Source: three-view drawing plus pictorial views. Frame: mm from the lowest corner of the part. Give positions to 0.01 mm unless a question says otherwise; leave off trailing zeros. Loops run counter-clockwise (first coordinate to the right, second up) from the corner with the lowest first, then second, coordinate; pieces in that order, holes last. Notation, with made-up numbers: M -40,67.5 L -24,67.5 A28 ccw -24,86.5 Z; hole C 53,56 d7. An arc over 180 degrees is marked long. Answer as a JSON object with one key per item and string values. Group by question number.
1) Section query C-C on y = 10. Return loops of the section in (x, z).
2) Section query A-A on z = 352. Return loops of the section in (x, y), plus the area to 3 significant figures.
3) Ray query, L1, parallel to X at y = 13.5, z = 229.5; L2, parallel to Z at x = 1394, y = 34; L3, parallel to Z at x = 262, y = 25.5. Return the intervals inside material, ascending.
4) Section query B-B on x = 1876.5. Return loops of the section in (y, z).
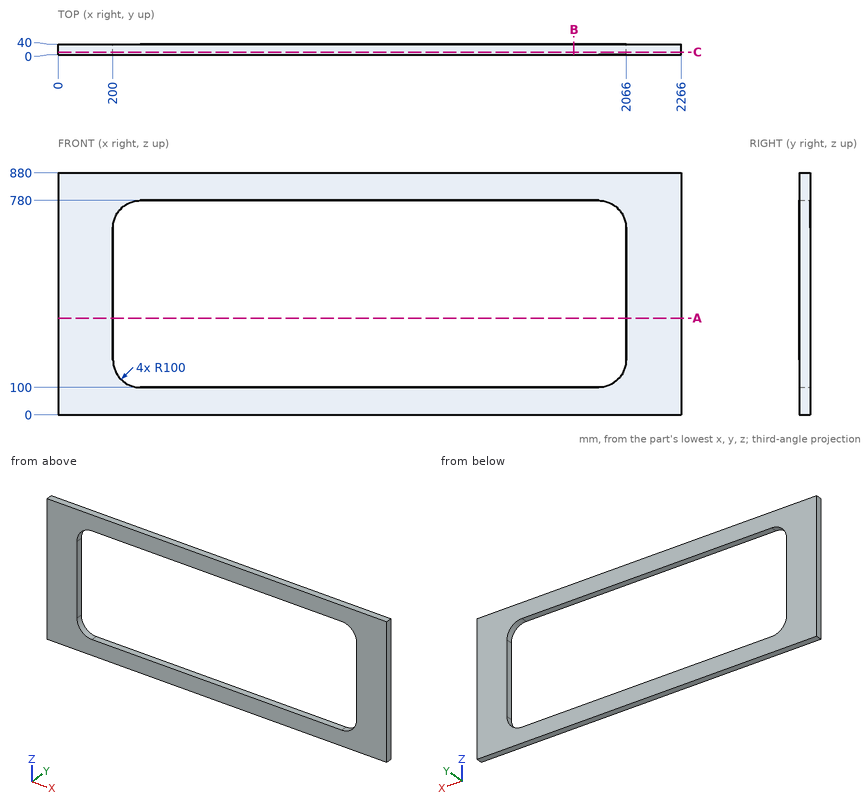
Output:
{
 "1": {"outline": "M 0,0 L 2266,0 L 2266,880 L 0,880 Z; hole M 200,200 A100 ccw 300,100 L 1966,100 A100 ccw 2066,200 L 2066,680 A100 ccw 1966,780 L 300,780 A100 ccw 200,680 Z"},
 "2": {"outline": "M 0,0 L 200,0 L 200,40 L 0,40 Z; M 2066,0 L 2266,0 L 2266,40 L 2066,40 Z", "area": "16,000 mm^2"},
 "3": {"L1": "x = 0 to 200, 2066 to 2266", "L2": "z = 0 to 100, 780 to 880", "L3": "z = 0 to 107.5, 772.5 to 880"},
 "4": {"outline": "M 0,0 L 40,0 L 40,100 L 0,100 Z; M 0,780 L 40,780 L 40,880 L 0,880 Z"}
}
